```python
from build123d import *

# Parameters (mm, degrees)
BOSS_EXTRUDE1_DEPTH  = 1
M6_CLEARANCE_HOLE1_D = 6.6
FILLET1_R            = 1


with BuildPart() as part:
    # Sketch1 → Boss-Extrude1 (new body)
    with BuildSketch(Plane.XY):
        Polygon((2, 6), (6, 6), (6, -6), (-6, -6), (-6, 6), (-2, 6), (-2, 17), (2, 17), align=None)
    extrude(amount=BOSS_EXTRUDE1_DEPTH)

    # M6 Clearance Hole1 (through all)
    with Locations(Plane.XY.offset(1)):
        with Locations((0, 0)):
            Hole(M6_CLEARANCE_HOLE1_D / 2)

    # Fillet1
    fillet1_edges = [part.edges().sort_by_distance(p)[0] for p in [
        (6, -6, 0.5),
        (-6, -6, 0.5),
        (-6, 6, 0.5),
        (-2, 6, 0.5),
        (-2, 17, 0.5),
        (2, 17, 0.5),
        (2, 6, 0.5),
        (6, 6, 0.5),
    ]]
    fillet(fillet1_edges, radius=FILLET1_R)


solid = part.part
```
Can you work these out from the model? Positions are in its coordinate system, mm. A direction names the side the tool comes from. Coordinates: 2 decimals unless noted, no trailing zeros. Loops run counter-clockwise (first coordinate to the right, second up) from the corner with the lowest first, then second, coordinate; pieces in that order, holes last.
1) Imagine slicing it at C-C on z = 0.45. List the corners of the cut face in (x, y) for me.
2) Which directions (+Z, -Z, +X, -X, +Y, -Y) give clear straight access to the entire face, cutting with the end or side of a thin tool? Please do faces 4 (the flat face through (0.1, -6, 0.5)), 5 (the flat face through (2, 11.6, 0.5)), 6 (the flat face through (-4, 6, 0.5)).
3) Imagine slicing it at A-A on y = 0. List the corners of the cut face in (x, z) for me, plus the area to 3 significant figures.
4) Imagine slicing it at B-B on x = 0. List the corners of the cut face in (y, z) for me.
5) Imagine slicing it at D-D on y = 12.75. List the corners of the cut face in (x, z) for me, plus the area to 3 significant figures.
6) I need wall thicknesses on probe 1 along Y at (x, z) = (0, 0.55); probe 2 along Y at (x, z) = (-1.5, 0.3); probe 3 along X at (y, z) = (7, 0.45). Which ranges of each line are inside material? Lowest first, please.
7) Thinking about a two-plate mould opening in X: for faces 1 (the cylindrical face through (2.301, 6.285, 0.507)), 2 (the flat face through (0, 17, 0.5)), 3 (the cylindrical face through (2.43, 2.23, 0.49)), which applies, pulls with the +X half, pulls with the -X half, needs draft (parallel to the pull), parting line crosses it, or undercut?
Completed:
1. outline: (-6, -5) arc R1 ccw to (-5, -6) - (5, -6) arc R1 ccw to (6, -5) - (6, 5) arc R1 ccw to (5, 6) - (3, 6) arc R1 cw to (2, 7) - (2, 16) arc R1 ccw to (1, 17) - (-1, 17) arc R1 ccw to (-2, 16) - (-2, 7) arc R1 cw to (-3, 6) - (-5, 6) arc R1 ccw to (-6, 5) - close; hole circle Ø6.6 at (0, 0)
2. face 4: +Z, -Z, +X, -X, -Y
2. face 5: +Z, -Z, +X, +Y
2. face 6: +Z, -Z, -X, +Y
3. outline: (-6, 0) - (-3.3, 0) - (-3.3, 1) - (-6, 1) - close; (3.3, 0) - (6, 0) - (6, 1) - (3.3, 1) - close
3. area: 5.40 mm2
4. outline: (-6, 0) - (-3.3, 0) - (-3.3, 1) - (-6, 1) - close; (3.3, 0) - (17, 0) - (17, 1) - (3.3, 1) - close
5. outline: (-2, 0) - (2, 0) - (2, 1) - (-2, 1) - close
5. area: 4.00 mm2
6. probe 1: y = -6 to -3.3, 3.3 to 17
6. probe 2: y = -6 to -2.94, 2.94 to 16.87
6. probe 3: x = -2 to 2
7. face 1: pulls with the +X half
7. face 2: needs draft
7. face 3: undercut
